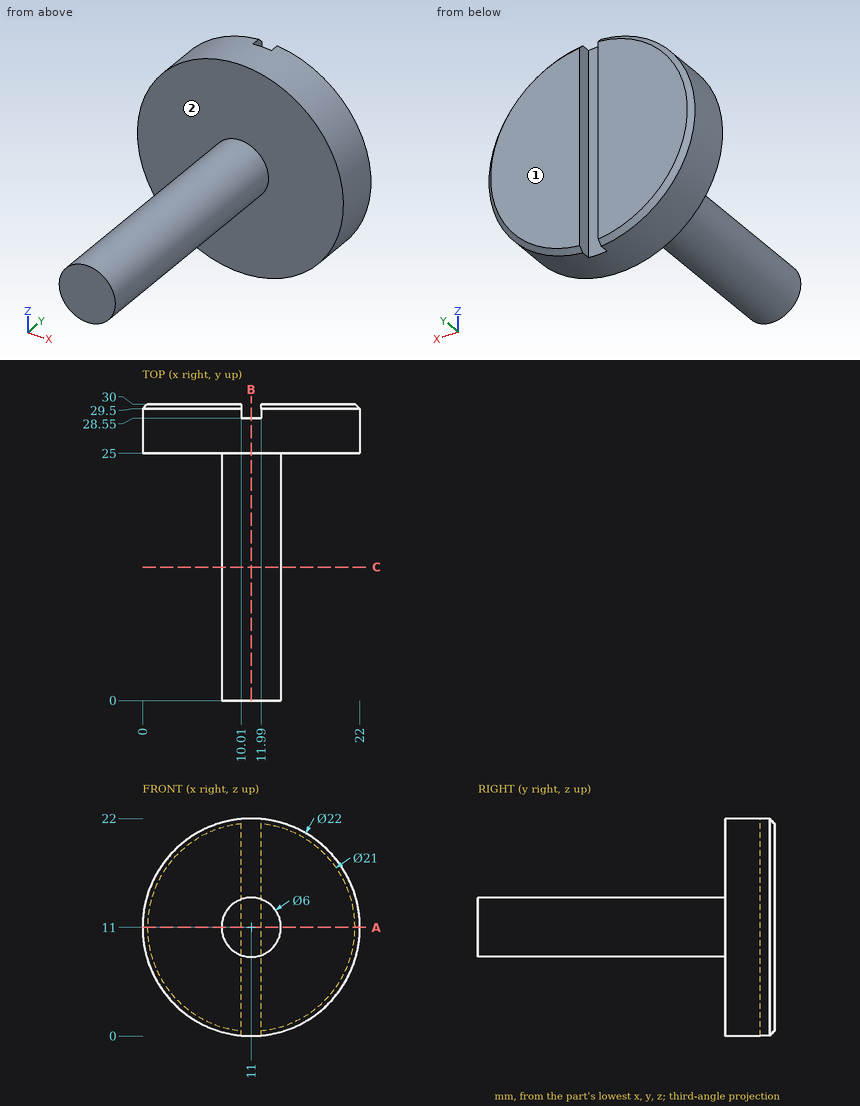
Drawing for the job (mm, zero at the part's lowest x, y, z). A direction names the side the tool comes from. Coordinates: 2 decimals unless noted, no trailing zeros. Order: outer loops, then holes, each group sorted by start corner. A loop starts at its lowest first (then second) coordinate and runs counter-clockwise, first axis right, second up. Notation, with made-up numbers: (63.25, 67.5) - (107.25, 67.5) arc R21 cw to (107.25, 99.5) - close; hole circle Ø2 at (-30, 31.5). An arc over 180 degrees is marked (long way). Use a Markdown table: item, result. Add a question column.
(1) Which spindle directions (+Z, -Z, +X, -X, +Y, -Y) get a long thin tool onto all of the face, cutting with end or side? Do the marked faces 1 and 2. Say none if no direction does.
(2) Saw through at B-B (x = 11). Give the cut face in (y, z), then the cut area to 3 significant figures.
(3) Drill centre lines: line 1 along Y through (x, z) = (16.25, 7.5); line 2 along Y through (x, z) = (10.25, 6); line 3 along X through (y, z) = (14.5, 13). Where is each one in solid material? Low to high. Write a range as [from, to].
(4) Saw through at A-A (z = 11). Give the cut face in (x, y).
(5) Saw through at C-C (y = 13.5). Give the cut face in (x, z).
(6) Flat gauge pins, fed straight in: pin 1 (12 mm diameter, centred on y = 13, z = 9, fed in from +X); pin 2 (1.5 mm diameter, centred on y = 27, z = 5.5, fed in from -X); pin 3 (4 mm diameter, centred on x = 7.5, y = 14, fed in from +Z). Where does each tip first touch, or does it go through?
Solved:
| question | item | result |
|---|---|---|
| 1 | face 1 | +Z, -Z, +X, -X, +Y |
| 1 | face 2 | -Y |
| 2 | outline | (0, 8) - (25, 8) - (25, 0) - (28.55, 0) - (28.55, 22) - (25, 22) - (25, 14) - (0, 14) - close |
| 2 | area | 228 mm² |
| 3 | line 1 | y = [25, 30] |
| 3 | line 2 | y = [25, 28.55] |
| 3 | line 3 | x = [8.76, 13.24] |
| 4 | outline | (0, 25) - (8, 25) - (8, 0) - (14, 0) - (14, 25) - (22, 25) - (22, 29.5) - (21.5, 30) - (11.99, 30) - (11.99, 28.55) - (10.01, 28.55) - (10.01, 30) - (0.5, 30) - (0, 29.5) - close |
| 5 | outline | circle Ø6 at (11, 11) |
| 6 | pin 1 | stops at x = 14 |
| 6 | pin 2 | stops at x = 1.08 |
| 6 | pin 3 | stops at z = 13.6 |
